from build123d import *

# Parameters (mm, degrees)
SKETCH1_W           = 440
SKETCH1_H           = 90
BOSS_EXTRUDE1_DEPTH = 40
M20_TAPPED_HOLE1_D  = 17.5


with BuildPart() as part:
    # Sketch1 → Boss-Extrude1 (new body)
    with BuildSketch(Plane.XY):
        with Locations((220, 45)):
            Rectangle(SKETCH1_W, SKETCH1_H)
    extrude(amount=BOSS_EXTRUDE1_DEPTH)

    # M20 Tapped Hole1 (through all)
    with Locations(Plane.XY.offset(40)):
        with Locations((36, 45), (404, 45)):
            Hole(M20_TAPPED_HOLE1_D / 2)


solid = part.part
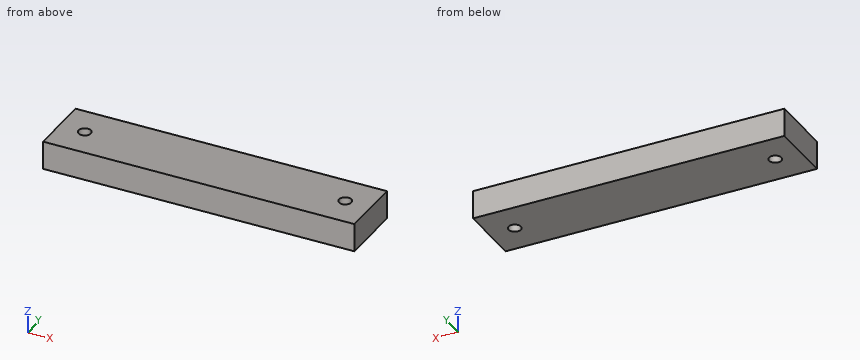
Verification items for the finished model (mm, model axes). Coordinates: 2 decimals unless noted, no trailing zeros. Loops run counter-clockwise (first coordinate to the right, second up) from the corner with the lowest first, then second, coordinate; pieces in that order, holes last. Notation, with made-up numbers: (82, 9.5) -> (98, 9.5) arc R17 ccw to (98, 20.5) -> close; hole circle Ø8 at (12.5, 58.5). An arc over 180 degrees is marked (long way). Write each question's results on one line, items separated by ' | '.
Item 1: Section check B-B, the plane x = 36. Enter the section's corners in (y, z).
Found:
outline: (0, 0) -> (36.25, 0) -> (36.25, 40) -> (0, 40) -> close; (53.75, 0) -> (90, 0) -> (90, 40) -> (53.75, 40) -> close
Item 2: Section check A-A, the plane y = 45. Enter the section's corners in (x, z), plus the area to 3 significant figures.
Found:
outline: (0, 0) -> (27.25, 0) -> (27.25, 40) -> (0, 40) -> close; (44.75, 0) -> (395.25, 0) -> (395.25, 40) -> (44.75, 40) -> close; (412.75, 0) -> (440, 0) -> (440, 40) -> (412.75, 40) -> close | area: 16,200 mm2
Item 3: Material ranges on L1, parallel to Y at x = 404, z = 30; L2, parallel to X at y = 42, z = 12; L3, parallel to X at y = 53, z = 33.5, recorded low to high.
Found:
L1: y = 0 to 36.25, 53.75 to 90 | L2: x = 0 to 27.78, 44.22 to 395.78, 412.22 to 440 | L3: x = 0 to 32.46, 39.54 to 400.46, 407.54 to 440
